Here's the drawing with two shaded views (mm, measured from the low corner). I have some questions. Round coordinates to 2 decimals unless told otherwise and drop trailing zeros. Loops run counter-clockwise (first coordinate to the right, second up) from the corner with the lowest first, then second, coordinate; pieces in that order, holes last. Notation, with made-up numbers: (18, -37.75) - (67, -37.75) arc R35 cw to (67, -5.75) - close; hole circle Ø2 at (-39, 23). An arc over 180 degrees is marked (long way). Use one line per item in the form item = value.
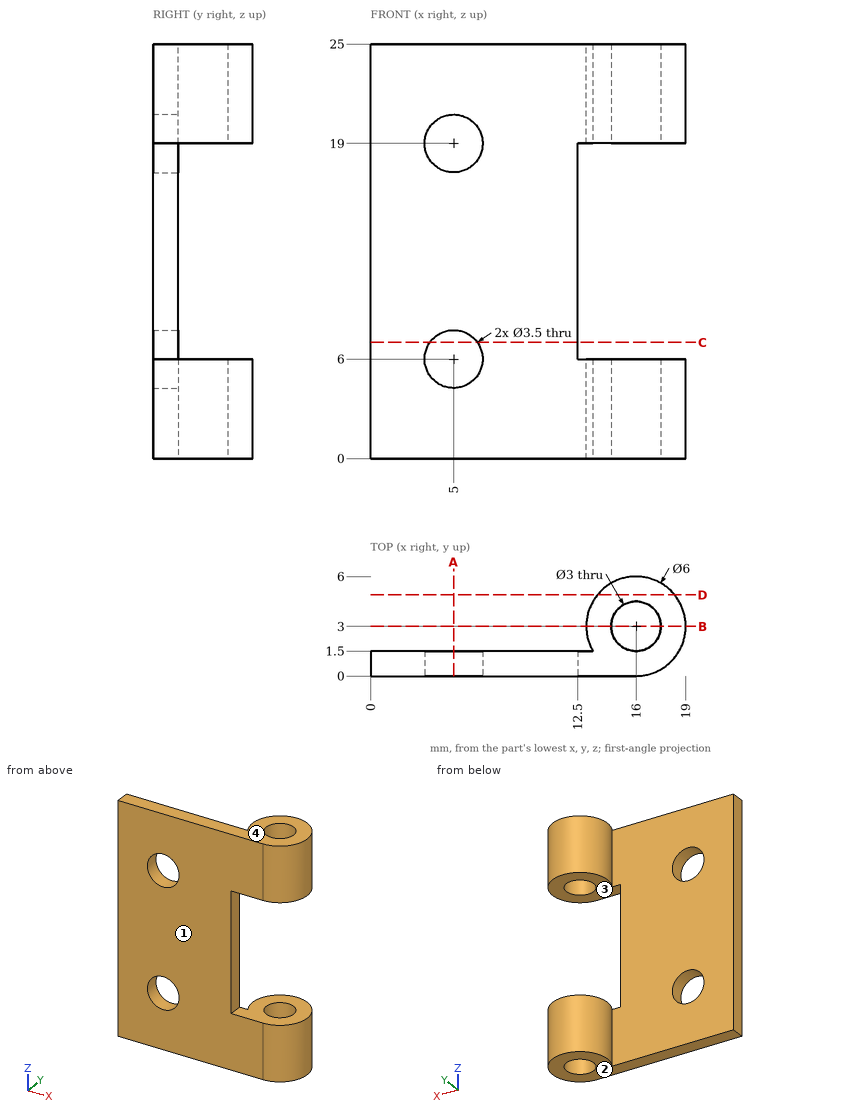
1. If we section it at D-D, the plane y = 4.9: Write out the boundary of the cut face in (x, z), plus the area to 3 significant figures.
Solution:
outline = (13.68, 0) - (18.32, 0) - (18.32, 6) - (13.68, 6) - close; (13.68, 19) - (18.32, 19) - (18.32, 25) - (13.68, 25) - close
area = 55.7 mm^2
2. If we section it at C-C, the plane z = 7: Write out the boundary of the cut face in (x, y), plus the area to 3 significant figures.
Solution:
outline = (0, 0) - (3.56, 0) - (3.56, 1.5) - (0, 1.5) - close; (6.44, 0) - (12.5, 0) - (12.5, 1.5) - (6.44, 1.5) - close
area = 14.4 mm^2
3. If we section it at A-A, the plane x = 5: Write out the boundary of the cut face in (y, z).
Solution:
outline = (0, 0) - (1.5, 0) - (1.5, 4.25) - (0, 4.25) - close; (0, 7.75) - (1.5, 7.75) - (1.5, 17.25) - (0, 17.25) - close; (0, 20.75) - (1.5, 20.75) - (1.5, 25) - (0, 25) - close
4. We'd pull the mould along Z, two halves only. Please class the marked faces 1, 2, 3 and 4: +Z half, -Z half, draft (parallel to the pull), parting line (faces both ways), or undercut.
Solution:
face_1 = draft
face_2 = -Z half
face_3 = undercut
face_4 = +Z half
5. If we section it at B-B, the plane y = 3: Write out the boundary of the cut face in (x, z).
Solution:
outline = (13, 0) - (14.5, 0) - (14.5, 6) - (13, 6) - close; (13, 19) - (14.5, 19) - (14.5, 25) - (13, 25) - close; (17.5, 0) - (19, 0) - (19, 6) - (17.5, 6) - close; (17.5, 19) - (19, 19) - (19, 25) - (17.5, 25) - close
6. Please list where these lines run through material, in increasing order: line 1 along Z through (x, y) = (5, 0.8); line 2 along Z through (x, y) = (14.25, 2.1); line 3 along X through (y, z) = (3, 22.45).
Solution:
line_1 = 0 to 4.25, 7.75 to 17.25, 20.75 to 25
line_2 = 0 to 6, 19 to 25
line_3 = 13 to 14.5, 17.5 to 19
7. For P1, Ø0.8, axis at y = 1, z = 14.5, coming from the +X side; P2, Ø1, axis at x = 2, z = 20.5, coming from the +Y side; P3, Ø1, axis at x = 10.5, z = 21, coming from the -Y side; P4, Ø1, axis at y = 3, z = 19, coming from the -X side, each with a flat end and sliding along its axis, tell me the tip position at first contact or that it passes through.
Solution:
P1 = 12.5
P2 = 1.5
P3 = 0
P4 = 13
